Source: CAD feature listing. Evaluate the final solid. Frame: model axes, mm. A direction names the side the tool comes from. Round coordinates to 2 decimals unless told otherwise and drop trailing zeros. Order: outer loops, then holes, each group sorted by start corner. A loop starts at its lowest first (then second) coordinate and runs counter-clockwise, first axis right, second up. Notation, with made-up numbers: M -37.5,0.25 L -28.5,0.25 A6 ccw -28.5,6.25 Z; hole C 58,-33.5 d11. An arc over 180 degrees is marked long. Answer in a Markdown table with one row per item. Add a question column.
```python
from build123d import *

# Parameters (mm, degrees)
SKETCH1_R           = 2.6
SKETCH1_R_2         = 5
BOSS_EXTRUDE1_DEPTH = 5


with BuildPart() as part:
    # Sketch1 → Boss-Extrude1 (new body)
    with BuildSketch(Plane.XY):
        with BuildLine():
            Line((-72.991378041, -0.434123458), (0, 7.5))
            ThreePointArc((0, 7.5), (6.214243254, 4.199188109), (6.958607035, -2.79781846))
            Line((6.958607035, -2.79781846), (-12.355075838, -50.833933534))
            ThreePointArc((-12.355075838, -50.833933534), (-17.316674975, -55.265358427), (-23.849430907, -54.009136903))
            Line((-23.849430907, -54.009136903), (-76.716654152, -13.863225709))
            ThreePointArc((-76.716654152, -13.863225709), (-79.407988086, -5.885388122), (-72.991378041, -0.434123458))
        make_face()
        Circle(SKETCH1_R, mode=Mode.SUBTRACT)
        with Locations((-19.313682873, -48.036115074)):
            Circle(SKETCH1_R, mode=Mode.SUBTRACT)
        with Locations((-72.180906117, -7.89020388)):
            Circle(SKETCH1_R_2, mode=Mode.SUBTRACT)
        with BuildLine():
            Line((-7.969347023, -3.889011646), (-59.380826719, -9.508878151))
            ThreePointArc((-59.380826719, -9.508878151), (-61.090881727, -10.963000514), (-60.373031081, -13.089840994))
            Line((-60.373031081, -13.089840994), (-22.717890398, -41.684116257))
            ThreePointArc((-22.717890398, -41.684116257), (-20.97582215, -42.019108663), (-19.652729047, -40.837395359))
            Line((-19.652729047, -40.837395359), (-5.896390033, -6.623253591))
            ThreePointArc((-5.896390033, -6.623253591), (-6.1582725, -4.668875059), (-7.969347023, -3.889011646))
        make_face(mode=Mode.SUBTRACT)
    extrude(amount=BOSS_EXTRUDE1_DEPTH)


solid = part.part
```
(1) Line query: line 1 (Y direction, x = -17, z = 4.5); line 2 (Y direction, x = -6.5, z = 4.15); line 3 (X direction, y = -14, z = 4.8). Output: solid intervals per line, ascending. Write a range as from..to.
(2) Cut plane A-A (z = 2.8). Return loops of the section in (x, y).
(3) Cut plane C-C (y = -16). Return loops of the section in (x, z).
(4) Cut plane B-B (x = -34.5). Return loops of the section in (y, z).
(5) Access query for faces 4 (the face through (-17.22, -55.24, 2.46)), 5 (the face through (-61.08, -10.93, 2.46)). Directions: +Z, -Z, +X, -X, +Y, -Y. A direction counts if a zero-diameter tool reaches every point of the face in a straight line with its end or side. Return the directions, or none.
(6) Pin query (flat end, axial travel): pin 1 (8 mm diameter, centred on x = -2, y = -30, fed in from -Z); pin 2 (2 mm diameter, centred on y = -24.5, z = 2.5, fed in from -X). Return the tip coordinate at first contact, or that it passes through.
(7) Draft query along Y for faces 1 (the face through (-6.14, -4.69, 2.46)), 2 (the face through (-26, -3, 0)), 3 (the face through (6.16, 4.28, 2.46)). Return one class per face: +Y half, -Y half, draft (parallel to the pull), parting line (faces both ways), or undercut.
Answer list:
| question | item | result |
|---|---|---|
| 1 | line 1 | -55.17..-49.22, -46.85..-34.24, -4.88..5.65 |
| 1 | line 2 | -36.27..-8.12, -4.32..6.79 |
| 1 | line 3 | -76.54..-59.17, -8.86..2.45 |
| 2 | outline | M -76.72,-13.86 L -23.85,-54.01 A7.5 ccw -12.36,-50.83 L 6.96,-2.8 A7.5 ccw 0,7.5 L -72.99,-0.43 A7.5 ccw Z; hole C -72.18,-7.89 d10; hole M -60.37,-13.09 L -22.72,-41.68 A2 ccw -19.65,-40.84 L -5.9,-6.62 A2 ccw -7.97,-3.89 L -59.38,-9.51 A2 ccw Z; hole C -19.31,-48.04 d5.2; hole C 0,0 d5.2 |
| 3 | outline | M -73.9,0 L -56.54,0 L -56.54,5 L -73.9,5 Z; M -9.67,0 L 1.65,0 L 1.65,5 L -9.67,5 Z |
| 4 | outline | M -45.92,0 L -32.74,0 L -32.74,5 L -45.92,5 Z; M -6.79,0 L 3.75,0 L 3.75,5 L -6.79,5 Z |
| 5 | face 4 | +Z, -Z, -Y |
| 5 | face 5 | +Z, -Z |
| 6 | pin 1 | z = 0 |
| 6 | pin 2 | x = -64.03 |
| 7 | face 1 | undercut |
| 7 | face 2 | draft |
| 7 | face 3 | parting line |
